Could you check a few things on this model? Use its own coordinates, in mm. A direction names the side the tool comes from. Round coordinates to 2 decimals unless told otherwise and drop trailing zeros. Loops run counter-clockwise (first coordinate to the right, second up) from the corner with the lowest first, then second, coordinate; pieces in that order, holes last. Notation, with made-up numbers: M -1.75,4.25 L 38.25,4.25 A27 ccw 38.25,22.25 Z; hole C 25,37 d4. An arc over 180 degrees is marked long. Answer in a Markdown table with one row per item.
```python
from build123d import *

# Parameters (mm, degrees)
BOSS_EXTRUDE1_DEPTH = 4


with BuildPart() as part:
    # Sketch1 → Boss-Extrude1 (new, symmetric)
    with BuildSketch(Plane.XY):
        with BuildLine():
            Line((0, 12), (40, 12))
            ThreePointArc((40, 12), (52, 0), (40, -12))
            Line((40, -12), (0, -12))
            ThreePointArc((0, -12), (-12, 0), (0, 12))
        make_face()
        with BuildLine():
            Line((12, -5), (28, -5))
            ThreePointArc((28, -5), (29.414213562, -4.414213562), (30, -3))
            Line((30, -3), (30, 3))
            ThreePointArc((30, 3), (29.414213562, 4.414213562), (28, 5))
            Line((28, 5), (12, 5))
            ThreePointArc((12, 5), (10.585786438, 4.414213562), (10, 3))
            Line((10, 3), (10, -3))
            ThreePointArc((10, -3), (10.585786438, -4.414213562), (12, -5))
        make_face(mode=Mode.SUBTRACT)
    extrude(amount=BOSS_EXTRUDE1_DEPTH, both=True)

    # Sketch2 → M12 Tapped Hole1 (revolve, cut)
    with BuildSketch(Plane(origin=(0, 0, 4), x_dir=(0, -1, 0), z_dir=(1, 0, 0))):
        Polygon((0, 0), (0, 32.75), (5.1, 29.685610843), (5.1, 0.925), (6.025, 0), align=None)
    m12_tapped_hole1 = revolve(axis=Axis((0, 0, 10.35), (0, 0, -1)), mode=Mode.SUBTRACT)

    # Mirror1: M12 Tapped Hole1 across plane
    add(m12_tapped_hole1.mirror(Plane.XY), mode=Mode.SUBTRACT)

    # Mirror2: M12 Tapped Hole1 across plane
    add(m12_tapped_hole1.mirror(Plane(origin=(20, 0, 0), x_dir=(0, 0, 1), z_dir=(1, 0, 0))), mode=Mode.SUBTRACT)

    # Mirror2 copy 1 sketch → Mirror2 copy 1 (revolve, cut)
    with BuildSketch(Plane(origin=(40, 0, -4), x_dir=(0, -1, 0), z_dir=(-1, 0, 0))):
        Polygon((0, 0), (0, 32.75), (5.1, 29.685610843), (5.1, 0.925), (6.025, 0), align=None)
    revolve(axis=Axis((40, 0, -10.35), (0, 0, 1)), mode=Mode.SUBTRACT)


solid = part.part
```
1) I want a section at B-B, the plane z = 1. Please give me the cut outline in (x, y).
Computed:
| item | result |
|---|---|
| outline | M 0,-12 L 40,-12 A12 ccw 40,12 L 0,12 A12 ccw Z; hole C 0,0 d10.2; hole M 10,-3 A2 ccw 12,-5 L 28,-5 A2 ccw 30,-3 L 30,3 A2 ccw 28,5 L 12,5 A2 ccw 10,3 Z; hole C 40,0 d10.2 |
2) I want a section at C-C, the plane y = -8.75. Please give me the cut outline in (x, z), plus the area to 3 significant figures.
Computed:
| item | result |
|---|---|
| outline | M -8.21,-4 L 48.21,-4 L 48.21,4 L -8.21,4 Z |
| area | 451 mm² |
3) I need wall thicknesses on line 1 (X direction, y = 0, z = 1.5); line 2 (Y direction, x = 19.5, z = -1); line 3 (X direction, y = 4.25, z = -1.75). Which ranges of each line are inside material? Lowest first, please.
Computed:
| item | result |
|---|---|
| line 1 | x = -12 to -5.1, 5.1 to 10, 30 to 34.9, 45.1 to 52 |
| line 2 | y = -12 to -5, 5 to 12 |
| line 3 | x = -11.22 to -2.82, 2.82 to 10.44, 29.56 to 37.18, 42.82 to 51.22 |
4) I want a section at A-A, the plane y = 0. Please give me the cut outline in (x, z) (3 decimals), plus the area to 3 significant figures.
Computed:
| item | result |
|---|---|
| outline | M -12,-4 L -6.025,-4 L -5.1,-3.075 L -5.1,3.075 L -6.025,4 L -12,4 Z; M 5.1,-3.075 L 6.025,-4 L 10,-4 L 10,4 L 6.025,4 L 5.1,3.075 Z; M 30,-4 L 33.975,-4 L 34.9,-3.075 L 34.9,3.075 L 33.975,4 L 30,4 Z; M 45.1,-3.075 L 46.025,-4 L 52,-4 L 52,4 L 46.025,4 L 45.1,3.075 Z |
| area | 185 mm² |
5) If we mould it in two halves opening along Y, with no side actions, what happens to faces 3 (the face through (20, 12, 0)), 4 (the face through (52, 0, 0)), 5 (the face through (20.4, -5.2, -4)), 6 (the face through (10, 0, 0))? For each: released by +Y, released by -Y, zero draft, split by the parting line, or undercut.
Computed:
| item | result |
|---|---|
| face 3 | released by +Y |
| face 4 | split by the parting line |
| face 5 | zero draft |
| face 6 | undercut |
6) Which directions (+Z, -Z, +X, -X, +Y, -Y) give clear straight access to the entire face, cutting with the end or side of a thin tool? Please do faces 1 (the face through (29.4, -4.43, 0.06)), 2 (the face through (20.4, -5.2, 4)).
Computed:
| item | result |
|---|---|
| face 1 | +Z, -Z |
| face 2 | +Z, +X, -X, +Y, -Y |
7) Will these pins go through, and if not, where does the flat tip stop? P1, Ø4, axis at y = -6, z = 2, coming from the -X side; P2, Ø1.5, axis at x = -3.5, z = 0.5, coming from the -Y side; P3, Ø1.5, axis at y = 1, z = 2, coming from the +X side.
Computed:
| item | result |
|---|---|
| P1 | stops at x = -11.31 |
| P2 | stops at y = -11.68 |
| P3 | stops at x = 52 |
